from build123d import *

# Parameters (mm, degrees)
SKETCH1_R           = 2
BOSS_EXTRUDE1_DEPTH = 9
SKETCH2_W           = 37
SKETCH2_H           = 5
CUT_EXTRUDE1_DEPTH  = 9


with BuildPart() as part:
    # Sketch1 → Boss-Extrude1 (new body)
    with BuildSketch(Plane.XY):
        with BuildLine():
            Line((-20, 0), (20, 0))
            ThreePointArc((20, 0), (22.645751311, -5.791287847), (16.535898385, -4))
            Line((16.535898385, -4), (-16.535898385, -4))
            ThreePointArc((-16.535898385, -4), (-22.645751311, -5.791287847), (-20, 0))
        make_face()
        with Locations((20, -3.5)):
            Circle(SKETCH1_R, mode=Mode.SUBTRACT)
        with Locations((-20, -3.5)):
            Circle(SKETCH1_R, mode=Mode.SUBTRACT)
    extrude(amount=BOSS_EXTRUDE1_DEPTH)

    # Sketch2 → Cut-Extrude1 (cut)
    with BuildSketch(Plane(origin=(0, 0, 0), x_dir=(1, 0, 0), z_dir=(0, 1, 0))):
        with Locations((-23.5, -4.5)):
            Rectangle(SKETCH2_W, SKETCH2_H)
    cut_extrude1 = extrude(amount=-CUT_EXTRUDE1_DEPTH, mode=Mode.SUBTRACT)

    # Mirror1: Cut-Extrude1 across plane
    add(cut_extrude1.mirror(Plane(origin=(0, 0, 0), x_dir=(0, 0, 1), z_dir=(1, 0, 0))), mode=Mode.SUBTRACT)


solid = part.part
The listing builds one solid part. Answer for the finished solid, in the listing's coordinates (mm). A direction names the side the tool comes from. Give positions to 0.01 mm unless a question says otherwise; leave off trailing zeros. Order: outer loops, then holes, each group sorted by start corner. A loop starts at its lowest first (then second) coordinate and runs counter-clockwise, first axis right, second up. Notation, with made-up numbers: (48.5, -34) - (92.5, -34) arc R22 ccw to (92.5, -24) - close; hole circle Ø8 at (-34, 85.5). An arc over 180 degrees is marked (long way). Answer as CSV lines item,"result".
Q1. Straight lines are drawn through the part: L1, parallel to X at y = -3.5, z = 7.75; L2, parallel to Z at x = 12.5, y = -3.25; L3, parallel to Y at x = -20, z = 8.4. For each, find the intervals that lie inside material, in ascending order.
Answer key:
L1,"x = -23.5 to -22, -18 to 18, 22 to 23.5"
L2,"z = 0 to 2, 7 to 9"
L3,"y = -7 to -5.5, -1.5 to 0"
Q2. Determine the mould class of faces 1 (the face through (-22.571, -5.875, 0.986)), 2 (the face through (5, -2, 5)), 3 (the face through (14, -3, 2)), 4 (the face through (-22.571, -5.875, 7.986)) for opening direction X: pulls with the +X half, pulls with the -X half, needs draft (parallel to the pull), parting line crosses it, or undercut.
Answer key:
face 1,"undercut"
face 2,"pulls with the +X half"
face 3,"needs draft"
face 4,"undercut"
Q3. A cutting plane is placed at B-B, the plane y = -3.5. Determine the outline of the cut face in (x, z).
Answer key:
outline,"(-23.5, 0) - (-22, 0) - (-22, 2) - (-23.5, 2) - close; (-23.5, 7) - (-22, 7) - (-22, 9) - (-23.5, 9) - close; (-18, 0) - (18, 0) - (18, 2) - (5, 2) - (5, 7) - (18, 7) - (18, 9) - (-18, 9) - (-18, 7) - (-5, 7) - (-5, 2) - (-18, 2) - close; (22, 0) - (23.5, 0) - (23.5, 2) - (22, 2) - close; (22, 7) - (23.5, 7) - (23.5, 9) - (22, 9) - close"
Q4. A cutting plane is placed at A-A, the plane x = -14.5. Determine the outline of the cut face in (y, z).
Answer key:
outline,"(-4, 0) - (0, 0) - (0, 2) - (-4, 2) - close; (-4, 7) - (0, 7) - (0, 9) - (-4, 9) - close"
Q5. A cutting plane is placed at D-D, the plane x = 17. Determine the outline of the cut face in (y, z).
Answer key:
outline,"(-5.3, 0) - (0, 0) - (0, 2) - (-5.3, 2) - close; (-5.3, 7) - (0, 7) - (0, 9) - (-5.3, 9) - close"
Q6. Which of the six approach directions +Z, -Z, +X, -X, +Y, -Y give full straight-line access (tool end or side, diameter ignored) to faces 5 (the face through (0, -2, 9)), 6 (the face through (-21.6, -4.7, 8)), 7 (the face through (14, -3, 7)), 8 (the face through (0, -4, 4)), 9 (the face through (-5, -2, 5))?
Answer key:
face 5,"+Z, +X, -X, +Y, -Y"
face 6,"+Z, -Z"
face 7,"+X, +Y, -Y"
face 8,"+Z, -Z, -Y"
face 9,"-X, +Y, -Y"
Q7. A cutting plane is placed at C-C, the plane z = 1.5. Determine the outline of the cut face in (x, y), and give its area (3 significant figures).
Answer key:
outline,"(-20, 0) arc R3.5 ccw (long way) to (-16.54, -4) - (16.54, -4) arc R3.5 ccw (long way) to (20, 0) - close; hole circle Ø4 at (-20, -3.5); hole circle Ø4 at (20, -3.5)"
area,"189 mm^2"
Q8. Each of these flat-tipped pins is pushed along its axis until it touches: pin 1 Ø3 at (x, y) = (-20, -3.5) entering from +Z; pin 2 Ø4.5 at (x, z) = (6, 6) entering from -Y; pin 3 Ø3 at (y, z) = (-2.5, 4) entering from -X; pin 4 Ø3 at (x, z) = (-18, 7) entering from -Y. Where does it stop, or does it pass through?
Answer key:
pin 1,"passes through"
pin 2,"stops at y = -4"
pin 3,"stops at x = -5"
pin 4,"stops at y = -6.96"
